Here's the drawing with two shaded views (mm, measured from the low corner). I have some questions. A direction names the side the tool comes from. Coordinates: 2 decimals unless noted, no trailing zeros. Write each loop counter-clockwise with the first axis right and the second up, starting at its lowest first coordinate (ties: lowest second). Pieces come first, ordered by that corner, then holes.
Item 1: I'm going to push flat-ended pins straight in: pin 1 Ø8 at (y, z) = (23, 6.5) entering from +X; pin 2 Ø1.5 at (x, y) = (3.5, 67.5) entering from +Z; pin 3 Ø5 at (y, z) = (13, 13.5) entering from +X; pin 4 Ø1.6 at (x, z) = (15, 7) entering from +Y. Where does each tip first touch, or does it pass through?
Item 2: If we section it at A-A (z = 8): Please give me the cut outline in (x, y), then the cut area to 3 significant figures.
Item 3: If we section it at B-B (y = 89.5): Please give me the cut outline in (x, z).
Item 4: If we section it at C-C (z = 11.75): Please give me the cut outline in (x, y).
Item 5: For the marked faces 1, 2 and 3, which set-ups out of +Z, -Z, +X, -X, +Y, -Y let a thin tool reach every point of the face, with its end or its side?
Item 6: If I drill on line 1 (Y direction, x = 13.5, z = 6); line 2 (Z direction, x = 13, y = 11) (3 decimals), over which ranges is the centre line in solid material (lowest first)?
Item 7: If we section it at D-D (x = 4.25): Please give me the cut outline in (y, z).
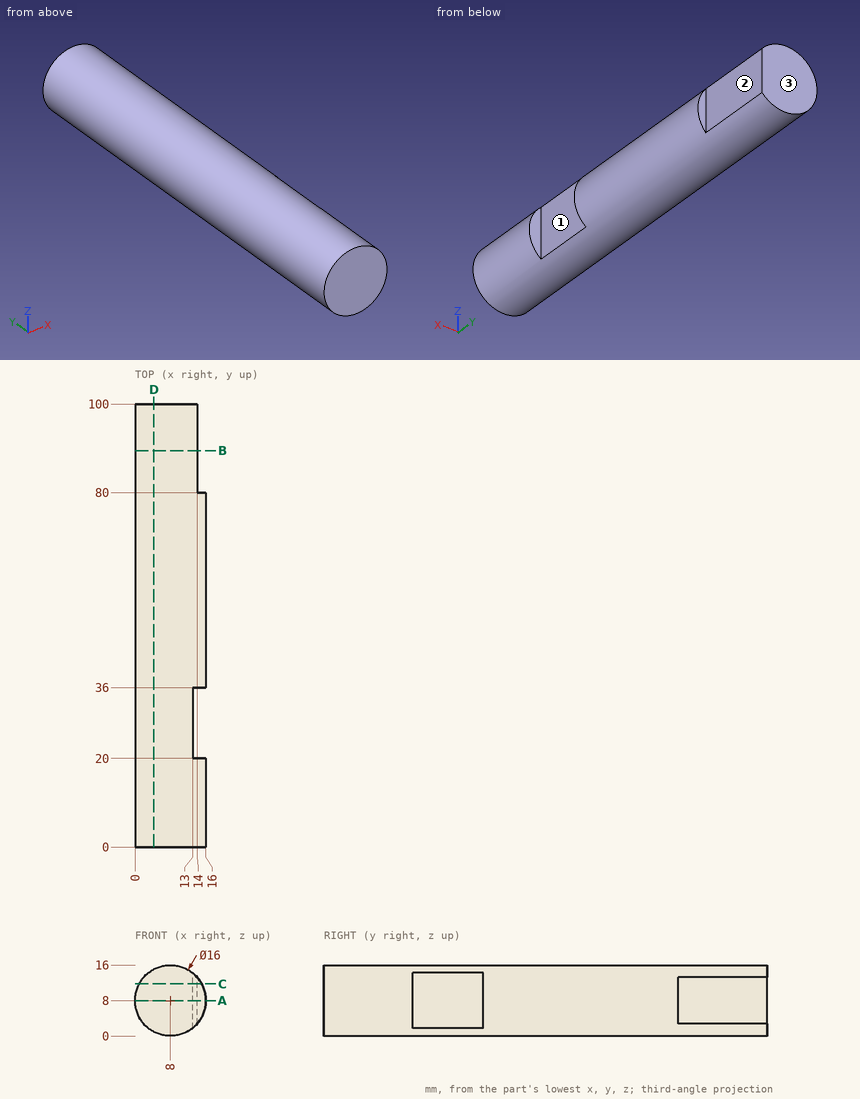
Answer list:
1. pin 1: stops at x = 16
1. pin 2: stops at z = 15.07
1. pin 3: stops at x = 15.42
1. pin 4: stops at y = 80
2. outline: (0, 0) - (16, 0) - (16, 20) - (13, 20) - (13, 36) - (16, 36) - (16, 80) - (14, 80) - (14, 100) - (0, 100) - close
2. area: 1,510 mm2
3. outline: (14, 2.71) - (14, 13.29) arc R8 ccw (long way) to start
4. outline: (0.93, 0) - (15.07, 0) - (15.07, 20) - (13, 20) - (13, 36) - (15.07, 36) - (15.07, 80) - (14, 80) - (14, 100) - (0.93, 100) - close
5. face 1: +Z, -Z, +X
5. face 2: +Z, -Z, +X, +Y
5. face 3: +Z, -Z, +X, -X, +Y
6. line 1: y = 0 to 20, 36 to 100
6. line 2: z = 1.755 to 14.245
7. outline: (0, 0.93) - (100, 0.93) - (100, 15.07) - (0, 15.07) - close
